```python
from build123d import *

# Parameters (mm, degrees)
SKETCH1_W                                           = 240
SKETCH1_H                                           = 24
BOSS_EXTRUDE1_DEPTH                                 = 8.5
CBORE_FOR_M4_HEX_SOCKET_HEAD_CAP_SCREW1_D           = 4.5
CBORE_FOR_M4_HEX_SOCKET_HEAD_CAP_SCREW1_CBORE_D     = 8
CBORE_FOR_M4_HEX_SOCKET_HEAD_CAP_SCREW1_CBORE_DEPTH = 4.4
LPATTERN1_COUNT                                     = 6
LPATTERN1_PITCH                                     = 40


with BuildPart() as part:
    # Sketch1 → Boss-Extrude1 (new body)
    with BuildSketch(Plane.XY):
        Rectangle(SKETCH1_W, SKETCH1_H)
    extrude(amount=BOSS_EXTRUDE1_DEPTH)

    # CBORE for M4 Hex Socket Head Cap Screw1 (through all)
    with Locations(Plane.XY.offset(8.5)):
        with Locations((-100, 0)):
            cbore_for_m4_hex_socket_head_cap_screw1 = CounterBoreHole(CBORE_FOR_M4_HEX_SOCKET_HEAD_CAP_SCREW1_D / 2, CBORE_FOR_M4_HEX_SOCKET_HEAD_CAP_SCREW1_CBORE_D / 2, CBORE_FOR_M4_HEX_SOCKET_HEAD_CAP_SCREW1_CBORE_DEPTH)

    # LPattern1: CBORE for M4 Hex Socket Head Cap Screw1 ×6
    with Locations(*[(i * LPATTERN1_PITCH, 0, 0) for i in range(1, LPATTERN1_COUNT)]):
        add(cbore_for_m4_hex_socket_head_cap_screw1, mode=Mode.SUBTRACT)


solid = part.part
```
Geometry: final body of the model. Coordinates: model frame, mm. A direction names the side the tool comes from. Round coordinates to 2 decimals unless told otherwise and drop trailing zeros. Order: outer loops, then holes, each group sorted by start corner. A loop starts at its lowest first (then second) coordinate and runs counter-clockwise, first axis right, second up. Notation, with made-up numbers: M -34.5,40.5 L -8.5,40.5 A11 ccw -8.5,56.5 Z; hole C 44.25,71.5 d11. An arc over 180 degrees is marked long. Use one line per item in the form item = value. Start each with the question number.
Q1. Access query for faces 4 (the face through (-2, 0, 8.5)), 5 (the face through (-23.2, -2.4, 6.3)). Directions: +Z, -Z, +X, -X, +Y, -Y. A direction counts if a zero-diameter tool reaches every point of the face in a straight line with its end or side. Return the directions, or none.
Q2. Cut plane B-B (z = 5.75). Return loops of the section in (x, y).
Q3. Material intervals for line 1 (Y direction, x = -60, z = 6.6); line 2 (Y direction, x = -20, z = 2.6), sorted ascending. Write a range as [from, to].
Q4. Mould query, pull axis X, two halves, no side actions, for faces 1 (the face through (-2, 0, 0)), 2 (the face through (-120, 0, 4)), 3 (the face through (62, -2, 4.1)). Classes: +X half, -X half, draft (parallel to the pull), parting line (faces both ways), or undercut.
Q5. Cut plane A-A (x = -100). Return loops of the section in (y, z), and give its area (3 significant figures).
Q6. Cut plane C-C (y = 0). Count the separate pieces of the cut face and the enclosed holes in it, and give its area (3 significant figures).
Q7. Pin query (flat end, axial travel): pin 1 Ø4 at (x, y) = (-60.5, -1) entering from +Z. Return the tip coordinate at first contact, or that it passes through.
Geometry results:
q1.face_4 = +Z, +X, -X, +Y, -Y
q1.face_5 = +Z
q2.outline = M -120,-12 L 120,-12 L 120,12 L -120,12 Z; hole C -100,0 d8; hole C -60,0 d8; hole C -20,0 d8; hole C 20,0 d8; hole C 60,0 d8; hole C 100,0 d8
q3.line_1 = [-12, -4], [4, 12]
q3.line_2 = [-12, -2.25], [2.25, 12]
q4.face_1 = draft
q4.face_2 = -X half
q4.face_3 = undercut
q5.outline = M -12,0 L -2.25,0 L -2.25,4.1 L -4,4.1 L -4,8.5 L -12,8.5 Z; M 2.25,0 L 12,0 L 12,8.5 L 4,8.5 L 4,4.1 L 2.25,4.1 Z
q5.area = 150 mm^2
q6.separate_pieces = 7
q6.enclosed_holes = 0
q6.area = 1,720 mm^2
q7.pin_1 = 4.1
